```python
from build123d import *

# Parameters (mm, degrees)
BOSS_EXTRUDE1_DEPTH = 300
SHELL1_T            = -2
SKETCH2_W           = 120
SKETCH2_H           = 600
CUT_EXTRUDE1_DEPTH  = 2


with BuildPart() as part:
    # Sketch1 → Boss-Extrude1 (new, symmetric)
    with BuildSketch(Plane.XY):
        Polygon((0, 120), (120, 80), (120, 0), (0, 0), align=None)
    extrude(amount=BOSS_EXTRUDE1_DEPTH, both=True)

    # Shell1
    shell1_openings = [part.faces().sort_by_distance(p)[0] for p in [
        (0, 60, 0),
    ]]
    offset(amount=SHELL1_T, openings=shell1_openings, kind=Kind.INTERSECTION)

    # Sketch2 → Cut-Extrude1 (cut)
    with BuildSketch(Plane.XZ):
        with Locations((60, 0)):
            Rectangle(SKETCH2_W, SKETCH2_H)
    extrude(amount=-CUT_EXTRUDE1_DEPTH, mode=Mode.SUBTRACT)


solid = part.part
```
Build history of the part. All positions in model axes, mm. A direction names the side the tool comes from. Round coordinates to 2 decimals unless told otherwise and drop trailing zeros. Loops run counter-clockwise (first coordinate to the right, second up) from the corner with the lowest first, then second, coordinate; pieces in that order, holes last.
Item 1: Which spindle directions (+Z, -Z, +X, -X, +Y, -Y) get a long thin tool onto all of the face, cutting with end or side? Do faces 1 (the face through (60, 48, 298)), 2 (the face through (59.16, 100.28, 4.2)). Say none if no direction does.
Item 2: Saw through at C-C (x = 65). List the corners of the cut face in (y, z).
Item 3: Saw through at A-A (y = 48.5). List the corners of the cut face in (x, z), then the cut area to 3 significant figures.
Item 4: Saw through at B-B (z = -77). List the corners of the cut face in (x, y), then the cut area to 3 significant figures.
Item 5: Drill centre lines: line 1 along Z through (x, y) = (69.5, 58.5); line 2 along X through (y, z) = (23, 134.5); line 3 along Y through (x, z) = (15.5, 232). Where is each one in solid material? Low to high.
Item 6: Two-plate mould, pull along Z, no slides. Class faces 3 (the face through (61, 49, 300)), 4 (the face through (118, 41, 4)), 5 (the face through (58.17, 98.5, 4.17)), 6 (the face through (120, 42, 4)): released by +Z, released by -Z, zero draft, split by the parting line, or undercut.
Item 7: Pin check, flat tips, straight feed: P1, Ø10, axis at y = 46, z = -129, coming from the -X side; P2, Ø6, axis at x = 61, z = -159, coming from the -Y side; P3, Ø8, axis at x = 66.5, z = -109.5, coming from the -Y side. Stop position of each tip, or through.
Worked answers:
1. face 1: -X, -Y
1. face 2: +Z, -Z, +X, +Y
2. outline: (2, -300) - (98.33, -300) - (98.33, 300) - (2, 300) - (2, 298) - (96.23, 298) - (96.23, -298) - (2, -298) - close
3. outline: (0, -300) - (120, -300) - (120, 300) - (0, 300) - (0, 298) - (118, 298) - (118, -298) - (0, -298) - close
3. area: 1,670 mm2
4. outline: (0, 117.89) - (118, 78.56) - (118, 2) - (120, 2) - (120, 80) - (0, 120) - close
4. area: 405 mm2
5. line 1: z = -300 to -298, 298 to 300
5. line 2: x = 118 to 120
5. line 3: y = 112.73 to 114.83
6. face 3: released by +Z
6. face 4: undercut
6. face 5: undercut
6. face 6: zero draft
7. P1: stops at x = 118
7. P2: stops at y = 96.56
7. P3: stops at y = 94.39
